Source: CAD feature listing. Evaluate the final solid. Frame: model axes, mm. A direction names the side the tool comes from. Give positions to 0.01 mm unless a question says otherwise; leave off trailing zeros. Loops run counter-clockwise (first coordinate to the right, second up) from the corner with the lowest first, then second, coordinate; pieces in that order, holes last. Notation, with made-up numbers: M 61,50 L 115,50 A32 cw 115,81 Z; hole C 33,55 d5. An arc over 180 degrees is marked long. Write item = value, one per line.
from build123d import *
from build123d.topology import SkipClean

# Parameters (mm, degrees)
BOSS_EXTRUDE1_DEPTH = 280
FILLET1_R           = 50
BOSS_EXTRUDE3_START = -30
BOSS_EXTRUDE3_DEPTH = 30
CUT_EXTRUDE5_START  = -30
CUT_EXTRUDE5_DEPTH  = 30
BOSS_EXTRUDE4_DEPTH = 30
CUT_EXTRUDE6_DEPTH  = 30
BOSS_EXTRUDE5_DEPTH = 325
CUT_EXTRUDE7_REACH  = 708.824
SKETCH7_R           = 25


with BuildPart() as part:
    # Sketch1 → Boss-Extrude1 (new body)
    with BuildSketch(Plane.XY):
        with BuildLine():
            Line((130, 0), (-130, 0))
            ThreePointArc((-130, 0), (-144.142135624, 5.857864376), (-150, 20))
            Line((-150, 20), (-150, 490))
            Line((-150, 490), (-180, 490))
            Line((-180, 490), (-180, -30))
            Line((-180, -30), (180, -30))
            Line((180, -30), (180, 490))
            Line((180, 490), (150, 490))
            Line((150, 490), (150, 20))
            ThreePointArc((150, 20), (144.142135624, 5.857864376), (130, 0))
        make_face()
    extrude(amount=BOSS_EXTRUDE1_DEPTH)

    # Fillet1
    fillet1_edges = [part.edges().sort_by_distance(p)[0] for p in [
        (180, -30, 140),
        (-180, -30, 140),
    ]]
    fillet(fillet1_edges, radius=FILLET1_R)

    # Sketch4 → Boss-Extrude3 (add)
    with BuildSketch(Plane.ZY.offset(180).offset(BOSS_EXTRUDE3_START)):
        with BuildLine():
            Line((247.238052948, 490), (140, 490))
            Line((140, 490), (140, 400))
            Line((140, 400), (280, 400))
            ThreePointArc((280, 400), (271.554793551, 447.888790898), (247.238052948, 490))
        make_face()
        with BuildLine():
            Line((140, 400), (140, 490))
            Line((140, 490), (32.761947052, 490))
            ThreePointArc((32.761947052, 490), (8.445206449, 447.888790898), (0, 400))
            Line((0, 400), (140, 400))
        make_face()
        with BuildLine():
            Line((247.238052948, 490), (140, 490))
            Line((140, 490), (140, 400))
            Line((140, 400), (280, 400))
            ThreePointArc((280, 400), (271.554793551, 447.888790898), (247.238052948, 490))
        make_face()
        with BuildLine():
            Line((140, 400), (140, 490))
            Line((140, 490), (32.761947052, 490))
            ThreePointArc((32.761947052, 490), (8.445206449, 447.888790898), (0, 400))
            Line((0, 400), (140, 400))
        make_face()
        with BuildLine():
            Line((32.761947052, 490), (140, 490))
            Line((140, 490), (247.238052948, 490))
            ThreePointArc((247.238052948, 490), (140, 540), (32.761947052, 490))
        make_face()
    extrude(amount=BOSS_EXTRUDE3_DEPTH)

    # Sketch4<3> → Cut-Extrude5 (cut)
    with SkipClean():  # the faces are left unmerged after this step: merging them gives an invalid solid
        with BuildSketch(Plane.ZY.offset(180).offset(CUT_EXTRUDE5_START)):
            with BuildLine():
                Line((0, 490), (0, 400))
                ThreePointArc((0, 400), (8.445206449, 447.888790898), (32.761947052, 490))
                Line((32.761947052, 490), (0, 490))
            make_face()
            with BuildLine():
                ThreePointArc((247.238052948, 490), (271.554793551, 447.888790898), (280, 400))
                Line((280, 400), (280, 490))
                Line((280, 490), (247.238052948, 490))
            make_face()
        extrude(amount=CUT_EXTRUDE5_DEPTH, mode=Mode.SUBTRACT)

    # Sketch5 → Boss-Extrude4 (add)
    with SkipClean():  # the faces are left unmerged after this step: merging them gives an invalid solid
        with BuildSketch(Plane(origin=(180, 0, 0), x_dir=(0, 0, -1), z_dir=(1, 0, 0))):
            with BuildLine():
                Line((-280, 400), (0, 400))
                ThreePointArc((0, 400), (-140, 540), (-280, 400))
            make_face()
        extrude(amount=-BOSS_EXTRUDE4_DEPTH)

    # Sketch5<2> → Cut-Extrude6 (cut)
    with SkipClean():  # the faces are left unmerged after this step: merging them gives an invalid solid
        with BuildSketch(Plane(origin=(180, 0, 0), x_dir=(0, 0, -1), z_dir=(1, 0, 0))):
            with BuildLine():
                Line((-280, 490), (-280, 400))
                ThreePointArc((-280, 400), (-271.554793551, 447.888790898), (-247.238052948, 490))
                Line((-247.238052948, 490), (-280, 490))
            make_face()
            with BuildLine():
                ThreePointArc((-32.761947052, 490), (-8.445206449, 447.888790898), (0, 400))
                Line((0, 400), (0, 490))
                Line((0, 490), (-32.761947052, 490))
            make_face()
        extrude(amount=-CUT_EXTRUDE6_DEPTH, mode=Mode.SUBTRACT)

    # Sketch6 → Boss-Extrude5 (add)
    with SkipClean():  # the faces are left unmerged after this step: merging them gives an invalid solid
        with BuildSketch(Plane.XZ.offset(30)):
            with BuildLine():
                ThreePointArc((37.5, 140), (26.516504294, 166.516504294), (0, 177.5))
                Line((0, 177.5), (0, 102.5))
                ThreePointArc((0, 102.5), (26.516504294, 113.483495706), (37.5, 140))
            make_face()
            with BuildLine():
                Line((0, 102.5), (0, 177.5))
                ThreePointArc((0, 177.5), (-37.5, 140), (0, 102.5))
            make_face()
            with BuildLine():
                ThreePointArc((37.5, 140), (26.516504294, 166.516504294), (0, 177.5))
                Line((0, 177.5), (0, 102.5))
                ThreePointArc((0, 102.5), (26.516504294, 113.483495706), (37.5, 140))
            make_face()
            with BuildLine():
                Line((0, 102.5), (0, 177.5))
                ThreePointArc((0, 177.5), (-37.5, 140), (0, 102.5))
            make_face()
        extrude(amount=BOSS_EXTRUDE5_DEPTH)

    # Cut-Extrude7: up to this face of the body (flat: up to its plane)
    cut_extrude7_end = Plane(part.part.faces().sort_by_distance((180, 210, 140))[0])
    # Sketch7 → Cut-Extrude7 (cut, up to the picked face)
    with BuildSketch(Plane.ZY.offset(180), mode=Mode.PRIVATE) as cut_extrude7_sk1:
        with Locations(Location((140, 400, 0), (0, 0, 270))):
            Circle(SKETCH7_R)
    cut_extrude7_tool1 = split(extrude(cut_extrude7_sk1.sketch, amount=-CUT_EXTRUDE7_REACH, mode=Mode.PRIVATE), bisect_by=cut_extrude7_end, keep=Keep.BOTH, mode=Mode.PRIVATE)
    add(cut_extrude7_tool1.solids().sort_by(Axis((-180, 400, 140), (1, 0, 0)))[0], mode=Mode.SUBTRACT)


solid = part.part
1. Cut plane C-C, the plane y = 416.5. Return the cut outline in (x, z).
Derived:
outline = M -180,0.98 L -150,0.98 L -150,121.22 L -180,121.22 Z; M -180,158.78 L -150,158.78 L -150,279.02 L -180,279.02 Z; M 150,0.98 L 180,0.98 L 180,121.22 L 150,121.22 Z; M 150,158.78 L 180,158.78 L 180,279.02 L 150,279.02 Z
2. Cut plane B-B, the plane z = 124.5. Return the cut outline in (x, y).
Derived:
outline = M -180,20 A50 ccw -130,-30 L -34.15,-30 L -34.15,-355 L 34.15,-355 L 34.15,-30 L 130,-30 A50 ccw 180,20 L 180,380.38 L 150,380.38 L 150,20 A20 cw 130,0 L -130,0 A20 cw -150,20 L -150,380.38 L -180,380.38 Z; M -180,419.62 L -150,419.62 L -150,539.14 L -180,539.14 Z; M 150,419.62 L 180,419.62 L 180,539.14 L 150,539.14 Z
3. Pull-direction query (Y, two-part tool) for faces 4 (the flat face through (150, 284, 138)), 5 (the flat face through (2, 0, 138)), 6 (the cylindrical face through (164.79, 376.154, 147.509)), 7 (the cylindrical face through (-165.21, 376.154, 147.509)); classes: +Y half, -Y half, draft (parallel to the pull), parting line (faces both ways), or undercut.
Derived:
face_4 = draft
face_5 = +Y half
face_6 = undercut
face_7 = undercut
4. First-contact query: pin 1 Ø2 at (y, z) = (383, 123.5) entering from +X; pin 2 Ø6 at (x, z) = (-135, 51.5) entering from -Y; pin 3 Ø12 at (x, z) = (105, 99) entering from +Y. Flat tips, straight axial feed; report the tip coordinate or a pass-through.
Derived:
pin_1 = through
pin_2 = -29.96
pin_3 = 0
5. Material intervals for probe 1 along X at (y, z) = (433.5, 144); probe 2 along Z at (x, y) = (-168, 400); probe 3 along Y at (x, z) = (37.5, 189.5), sorted ascending. Write a range as from..to.
Derived:
probe_1 = -180..-150, 150..180
probe_2 = 0..115, 165..280
probe_3 = -30..0
6. Reachability of faces 1 (the flat face through (-150, 276, 138)), 2 (the cylindrical face through (-165.742, -14.964, 141.96)), 3 (the flat face through (-31, -30, 169)) from +Z, -Z, +X, -X, +Y, -Y: full face, straight path, thin tool, end or side. Return the list, or none.
Derived:
face_1 = +Z, -Z, +Y
face_2 = +Z, -Z, -X, -Y
face_3 = -Y
7. Cut plane D-D, the plane z = 18. Return the cut outline in (x, y), then the cut area to 3 significant figures.
Derived:
outline = M -180,20 A50 ccw -130,-30 L 130,-30 A50 ccw 180,20 L 180,468.67 L 150,468.67 L 150,20 A20 cw 130,0 L -130,0 A20 cw -150,20 L -150,468.67 L -180,468.67 Z
area = 38,000 mm²
8. Cut plane A-A, the plane y = 188.5. Return the cut outline in (x, z), then the cut area to 3 significant figures.
Derived:
outline = M -180,0 L -150,0 L -150,280 L -180,280 Z; M 150,0 L 180,0 L 180,280 L 150,280 Z
area = 16,800 mm²
